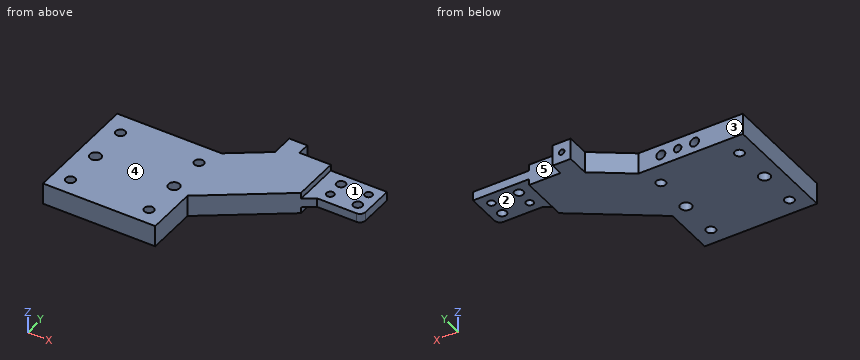
```python
from build123d import *

# Parameters (mm, degrees)
SKETCH1_R           = 4.188
SKETCH1_R_2         = 5
SKETCH1_R_3         = 3.3235
SKETCH1_R_4         = 4
BOSS_EXTRUDE1_DEPTH = 19
SKETCH2_R           = 4
SKETCH2_R_2         = 3.325
CUT_EXTRUDE1_DEPTH  = 15
SKETCH3_R           = 2.4585
CUT_EXTRUDE2_DEPTH  = 15
SKETCH4_W           = 50
SKETCH4_H           = 41.969696972
CUT_EXTRUDE3_DEPTH  = 5.5
SKETCH5_W           = 50
SKETCH5_H           = 41.969696972
CUT_EXTRUDE4_DEPTH  = 5.5
FILLET1_R           = 5


with BuildPart() as part:
    # Sketch1 → Boss-Extrude1 (new body)
    with BuildSketch(Plane.XY):
        Polygon((0, 0), (0, 104.0002829), (93, 104.0002829), (126, 127.0002829), (126, 147.0002829), (142, 147.0002829), (142, 136.0002829), (220, 136.0002829), (220, 101.000282896), (179.999999997, 101.000282896), (100, 45.24270714), (100, 0), align=None)
        with Locations((15, 15)):
            Circle(SKETCH1_R, mode=Mode.SUBTRACT)
        with Locations((15, 50)):
            Circle(SKETCH1_R_2, mode=Mode.SUBTRACT)
        with Locations((15, 85)):
            Circle(SKETCH1_R, mode=Mode.SUBTRACT)
        with Locations((85, 85)):
            Circle(SKETCH1_R, mode=Mode.SUBTRACT)
        with Locations((85, 50)):
            Circle(SKETCH1_R_2, mode=Mode.SUBTRACT)
        with Locations((85, 15)):
            Circle(SKETCH1_R, mode=Mode.SUBTRACT)
        with Locations((210.1, 125.7002829)):
            Circle(SKETCH1_R_3, mode=Mode.SUBTRACT)
        with Locations((210.1, 110.7002829)):
            Circle(SKETCH1_R_4, mode=Mode.SUBTRACT)
        with Locations((185.6, 110.7002829)):
            Circle(SKETCH1_R_3, mode=Mode.SUBTRACT)
        with Locations((185.6, 125.7002829)):
            Circle(SKETCH1_R_4, mode=Mode.SUBTRACT)
    extrude(amount=BOSS_EXTRUDE1_DEPTH)

    # Sketch2 → Cut-Extrude1 (cut)
    with BuildSketch(Plane(origin=(0, 104.0002829, 0), x_dir=(1, 0, 0), z_dir=(0, 1, 0))):
        with Locations(Location((43, -9.5, 0), (0, 0, 270))):
            Circle(SKETCH2_R)
        with Locations(Location((58, -9.5, 0), (0, 0, 270))):
            Circle(SKETCH2_R_2)
        with Locations(Location((73, -9.5, 0), (0, 0, 270))):
            Circle(SKETCH2_R)
    extrude(amount=-CUT_EXTRUDE1_DEPTH, mode=Mode.SUBTRACT)

    # Sketch3 → Cut-Extrude2 (cut)
    with BuildSketch(Plane(origin=(0, 147.0002829, 0), x_dir=(1, 0, 0), z_dir=(0, 1, 0))):
        with Locations(Location((134, -9.5, 0), (0, 0, 270))):
            Circle(SKETCH3_R)
    extrude(amount=-CUT_EXTRUDE2_DEPTH, mode=Mode.SUBTRACT)

    # Sketch4 → Cut-Extrude3 (cut)
    with BuildSketch(Plane.XY.offset(19)):
        with Locations((195, 115.015434414)):
            Rectangle(SKETCH4_W, SKETCH4_H)
    extrude(amount=-CUT_EXTRUDE3_DEPTH, mode=Mode.SUBTRACT)

    # Sketch5 → Cut-Extrude4 (cut)
    with BuildSketch(Plane(origin=(0, 0, 0), x_dir=(-1, 0, 0), z_dir=(0, 0, -1))):
        with Locations((-195, 115.015434414)):
            Rectangle(SKETCH5_W, SKETCH5_H)
    extrude(amount=-CUT_EXTRUDE4_DEPTH, mode=Mode.SUBTRACT)

    # Fillet1
    fillet1_edges = [part.edges().sort_by_distance(p)[0] for p in [
        (220, 101.000282896, 9.5),
    ]]
    fillet(fillet1_edges, radius=FILLET1_R)


solid = part.part
```
Input: part model. Units: mm. Frame: model coordinates. Face numbers are marked on the shaded views. A direction names the side the tool comes from. Give positions to 0.01 mm unless a question says otherwise; leave off trailing zeros. Order: outer loops, then holes, each group sorted by start corner. A loop starts at its lowest first (then second) coordinate and runs counter-clockwise, first axis right, second up.
1. Pin query (flat end, axial travel): pin 1 (6.5 mm diameter, centred on x = 43, z = 9.5, fed in from +Y); pin 2 (10.5 mm diameter, centred on x = 210.1, y = 125.7, fed in from +Z); pin 3 (1.5 mm diameter, centred on x = 145, z = 7.5, fed in from -Y). Return the tip coordinate at first contact, or that it passes through.
Derived:
pin 1: stops at y = 89
pin 2: stops at z = 13.5
pin 3: stops at y = 76.08
2. Material intervals for L1, parallel to Y at x = 85, z = 15; L2, parallel to X at y = 135, z = 9.25; L3, parallel to Y at x = 185.6, z = 9.5, sorted ascending.
Derived:
L1: y = 0 to 10.81, 19.19 to 45, 55 to 80.81, 89.19 to 104
L2: x = 126 to 131.55, 136.45 to 220
L3: y = 101 to 107.38, 114.02 to 121.7, 129.7 to 136
3. Section C-C on x = 58. Return the cut outline in (y, z) (3 decimals).
Derived:
outline: (0, 0) - (104, 0) - (104, 6.175) - (89, 6.175) - (89, 12.825) - (104, 12.825) - (104, 19) - (0, 19) - close
4. Section A-A on y = 15. Return the cut outline in (x, z).
Derived:
outline: (0, 0) - (10.81, 0) - (10.81, 19) - (0, 19) - close; (19.19, 0) - (80.81, 0) - (80.81, 19) - (19.19, 19) - close; (89.19, 0) - (100, 0) - (100, 19) - (89.19, 19) - close
5. Reachability of the marked faces 1, 2, 3, 4 and 5 from +Z, -Z, +X, -X, +Y, -Y: full face, straight path, thin tool, end or side. Return the list, or none.
Derived:
face 1: +Z, +X, +Y, -Y
face 2: -Z, +X, +Y, -Y
face 3: +Z, -Z, -X, +Y
face 4: +Z, +X, -X, +Y, -Y
face 5: +Z, -Z, +X, +Y
6. Section D-D on y = 50. Return the cut outline in (x, z), and give its area (3 significant figures).
Derived:
outline: (0, 0) - (10, 0) - (10, 19) - (0, 19) - close; (20, 0) - (80, 0) - (80, 19) - (20, 19) - close; (90, 0) - (106.83, 0) - (106.83, 19) - (90, 19) - close
area: 1,650 mm2
7. Section B-B on x = 85. Return the cut outline in (y, z).
Derived:
outline: (0, 0) - (10.81, 0) - (10.81, 19) - (0, 19) - close; (19.19, 0) - (45, 0) - (45, 19) - (19.19, 19) - close; (55, 0) - (80.81, 0) - (80.81, 19) - (55, 19) - close; (89.19, 0) - (104, 0) - (104, 19) - (89.19, 19) - close
